Geometry check sheet. Reference: drawing and pictorial views, mm from the part's lowest x, y, z. A direction names the side the tool comes from. Coordinates: 2 decimals unless noted, no trailing zeros. Loops run counter-clockwise (first coordinate to the right, second up) from the corner with the lowest first, then second, coordinate; pieces in that order, holes last. Notation, with made-up numbers: (27.5, 28) -> (84.5, 28) arc R33 ccw to (84.5, 66) -> close; hole circle Ø3 at (-18.75, 73). An arc over 180 degrees is marked (long way). Use one line per item in the form item = value.
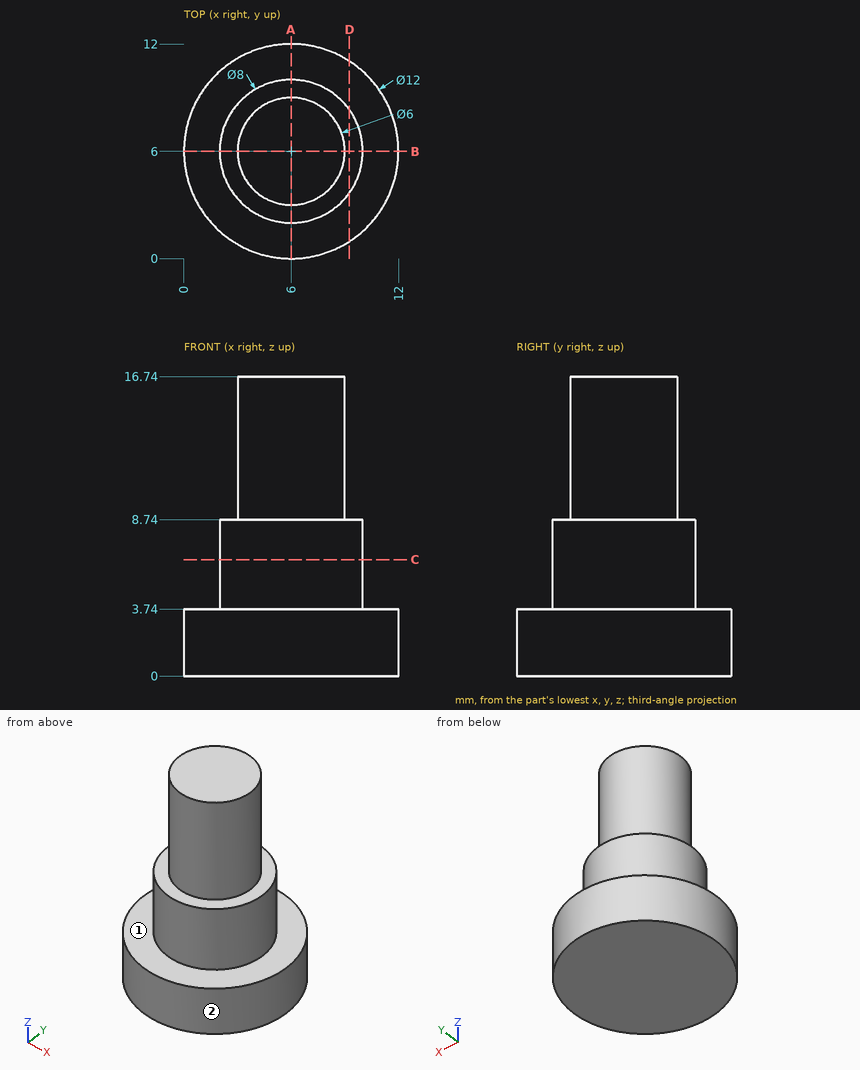
(1) Section check D-D, the plane x = 9.25. Record the boundary of the cut face in (y, z).
Established:
outline = (0.96, 0) -> (11.04, 0) -> (11.04, 3.74) -> (8.33, 3.74) -> (8.33, 8.74) -> (3.67, 8.74) -> (3.67, 3.74) -> (0.96, 3.74) -> close
(2) Go/stop test with flat-tipped pins: P1, Ø1, axis at y = 9.5, z = 6.5, coming from the -X side; P2, Ø2, axis at x = 5.5, z = 10.5, coming from the -Y side. Record where each tip stops, or that it passes through.
Established:
P1 = 3.35
P2 = 3
(3) Tool access check on the marked faces 1 and 2. Record the directions out of +Z, -Z, +X, -X, +Y, -Y that give a thin tool (end or side, any length) a straight path to the whole face; none if there is none.
Established:
face_1 = +Z
face_2 = +Z, -Z
(4) Scan lines: line 1 along Z through (x, y) = (3.75, 11.5); line 2 along Y through (x, z) = (6, 9.25); line 3 along Y through (x, z) = (6, 7.75). Record each from-to range of solid material in increasing order.
Established:
line_1 = 0 to 3.74
line_2 = 3 to 9
line_3 = 2 to 10
(5) Section check C-C, the plane z = 6.5. Record the boundary of the cut face in (x, y).
Established:
outline = circle Ø8 at (6, 6)
(6) Section check A-A, the plane x = 6. Record the boundary of the cut face in (y, z).
Established:
outline = (0, 0) -> (12, 0) -> (12, 3.74) -> (10, 3.74) -> (10, 8.74) -> (9, 8.74) -> (9, 16.74) -> (3, 16.74) -> (3, 8.74) -> (2, 8.74) -> (2, 3.74) -> (0, 3.74) -> close
